Job drawing, mm, ordinate dimensions from the low corner. One solid piece. Coordinates: 2 decimals unless noted, no trailing zeros. Order: outer loops, then holes, each group sorted by start corner. A loop starts at its lowest first (then second) coordinate and runs counter-clockwise, first axis right, second up. Notation, with made-up numbers: (60.25, 2.5) - (95.25, 2.5) arc R21 cw to (95.25, 30.5) - close; hole circle Ø2 at (-16.75, 20). An arc over 180 degrees is marked (long way). Write each question's results on one line, items separated by ' | '. Start each with the question number.
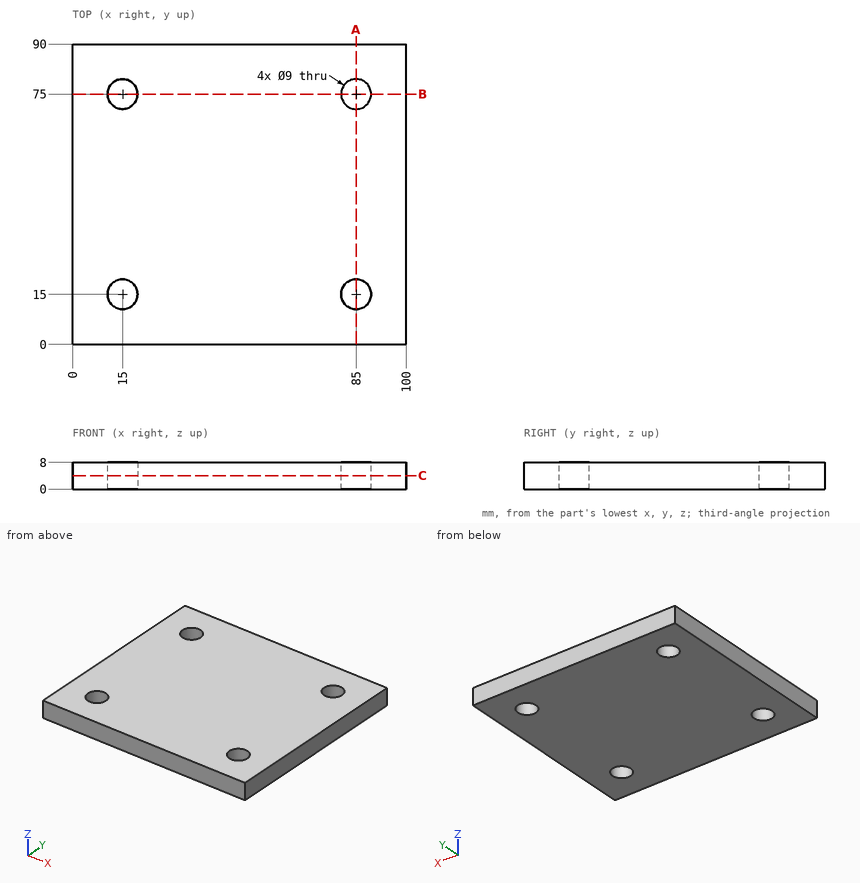
Item 1: Slice it at C-C (z = 4). Write the cut outline in (x, y), then the cut area to 3 significant figures.
Item 2: Probe probe 1 along X at (y, z) = (15, 6); probe 2 along Y at (x, z) = (85, 5.75); probe 3 along Y at (x, z) = (82, 3.5). List the from-to ranges inside material, lowest first.
Item 3: Slice it at B-B (y = 75). Write the cut outline in (x, z), then the cut area to 3 significant figures.
Item 4: Flat gauge pin, fed straight in: P1, Ø1.5, axis at y = 62.5, z = 3.5, coming from the -X side. Where does the tip first touch, or does it go through?
Item 5: Slice it at A-A (x = 85). Write the cut outline in (y, z).
Resolved:
1) outline: (0, 0) - (100, 0) - (100, 90) - (0, 90) - close; hole circle Ø9 at (15, 15); hole circle Ø9 at (15, 75); hole circle Ø9 at (85, 15); hole circle Ø9 at (85, 75) | area: 8,750 mm^2
2) probe 1: 0 to 10.5, 19.5 to 80.5, 89.5 to 100 | probe 2: 0 to 10.5, 19.5 to 70.5, 79.5 to 90 | probe 3: 0 to 11.65, 18.35 to 71.65, 78.35 to 90
3) outline: (0, 0) - (10.5, 0) - (10.5, 8) - (0, 8) - close; (19.5, 0) - (80.5, 0) - (80.5, 8) - (19.5, 8) - close; (89.5, 0) - (100, 0) - (100, 8) - (89.5, 8) - close | area: 656 mm^2
4) P1: x = 0
5) outline: (0, 0) - (10.5, 0) - (10.5, 8) - (0, 8) - close; (19.5, 0) - (70.5, 0) - (70.5, 8) - (19.5, 8) - close; (79.5, 0) - (90, 0) - (90, 8) - (79.5, 8) - close
